Source: CAD feature listing. Evaluate the final solid. Frame: model axes, mm. A direction names the side the tool comes from. Round coordinates to 2 decimals unless told otherwise and drop trailing zeros. Write each loop counter-clockwise with the first axis right and the second up, starting at its lowest first coordinate (ties: lowest second). Pieces come first, ordered by that corner, then holes. Notation, with made-up numbers: (82.5, 3) -> (122.5, 3) arc R12 cw to (122.5, 7) -> close; hole circle Ø7 at (-37.5, -30.5). An arc over 180 degrees is marked (long way). Put each result on its own line as item: value.
```python
from build123d import *

# Parameters (mm, degrees)
CHAMFER1_SIZE       = 1
CHAMFER2_SIZE       = 2
SKETCH2_OUTSIDE_W   = 53.512
SKETCH2_OUTSIDE_H   = 53.512
SKETCH2_OUTSIDE_W_2 = 10
SKETCH2_OUTSIDE_H_2 = 10
CUT_EXTRUDE1_DEPTH  = 35


with BuildPart() as part:
    # Sketch1 → Revolve1 (revolve)
    with BuildSketch(Plane.XY, mode=Mode.PRIVATE) as revolve1_sk:
        Polygon((0, 0), (0, 10), (80, 10), (80, 6), (155, 6), (155, 0), align=None)
    revolve(revolve1_sk.sketch.rotate(Axis((0, 0, 0), (1, 0, 0)), 90), axis=Axis((0, 0, 0), (1, 0, 0)))

    # Chamfer1
    chamfer1_edges = [part.edges().sort_by_distance(p)[0] for p in [
        (155, 0, -6),
    ]]
    chamfer(chamfer1_edges, length=CHAMFER1_SIZE)

    # Chamfer2
    chamfer2_edges = [part.edges().sort_by_distance(p)[0] for p in [
        (0, 0, -10),
    ]]
    chamfer(chamfer2_edges, length=CHAMFER2_SIZE)

    # Sketch2 outside → Cut-Extrude1 (cut)
    with BuildSketch(Plane(origin=(155, 0, 0), x_dir=(0, 0, -1), z_dir=(1, 0, 0))):
        Rectangle(SKETCH2_OUTSIDE_W, SKETCH2_OUTSIDE_H)
        Rectangle(SKETCH2_OUTSIDE_W_2, SKETCH2_OUTSIDE_H_2, mode=Mode.SUBTRACT)
    extrude(amount=-CUT_EXTRUDE1_DEPTH, mode=Mode.SUBTRACT)


solid = part.part
```
Q1. Draft query along Z for faces 1 (the conical face through (154.729, -3.686, 3.768)), 2 (the flat face through (0, 0, 0)), 3 (the cylindrical face through (109, 0, -6)), 4 (the conical face through (154.729, 3.686, -3.768)). Return one class per face: +Z half, -Z half, draft (parallel to the pull), parting line (faces both ways), or undercut.
Ans:
face 1: +Z half
face 2: draft
face 3: parting line
face 4: -Z half
Q2. Pin query (flat end, axial travel): pin 1 (6 mm diameter, centred on x = 16, y = -4.5, fed in from +Z); pin 2 (1.1 mm diameter, centred on y = 5.5, z = -1.5, fed in from +X); pin 3 (5 mm diameter, centred on x = 109, y = 6.5, fed in from -Z). Return the tip coordinate at first contact, or that it passes through.
Ans:
pin 1: stops at z = 9.89
pin 2: stops at x = 154.85
pin 3: stops at z = -4.47
Q3. Reachability of faces 5 (the flat face through (138, -5, 0)), 6 (the flat face through (138, 0, -5)), 7 (the flat face through (80, 0, 7)), 8 (the flat face through (138, 5, 0)) from +Z, -Z, +X, -X, +Y, -Y: full face, straight path, thin tool, end or side. Return the list, or none.
Ans:
face 5: +Z, -Z, +X, -Y
face 6: -Z, +X, +Y, -Y
face 7: +X
face 8: +Z, -Z, +X, +Y
Q4. Cut plane A-A on x = 48. Output: boundary loops of the cut face in (y, z), and give its area (3 significant figures).
Ans:
outline: circle Ø20 at (0, 0)
area: 314 mm^2
Q5. Material intervals for line 1 (Z direction, x = 130.5, y = 0.5); line 2 (X direction, y = 6.5, z = -1.75), sorted ascending. Write a range as [from, to].
Ans:
line 1: z = [-5, 5]
line 2: x = [0, 80]
